Build history of the part. All positions in model axes, mm. A direction names the side the tool comes from. Coordinates: 2 decimals unless noted, no trailing zeros. Write each loop counter-clockwise with the first axis right and the second up, starting at its lowest first coordinate (ties: lowest second). Pieces come first, ordered by that corner, then holes.
```python
from build123d import *

# Parameters (mm, degrees)
EXTRUDE_1_DEPTH = 7.5


with BuildPart() as part:
    # 草图1 → 凸台-拉伸1 (new, symmetric)
    with BuildSketch(Plane.XY):
        with BuildLine():
            Line((0, 14.17), (937, 14.17))
            ThreePointArc((937, 14.17), (951.17, 0), (937, -14.17))
            Line((937, -14.17), (0, -14.17))
            ThreePointArc((0, -14.17), (-14.17, 0), (0, 14.17))
        make_face()
        with BuildLine():
            Line((0, 12.99), (937, 12.99))
            ThreePointArc((937, 12.99), (949.99, 0), (937, -12.99))
            Line((937, -12.99), (0, -12.99))
            ThreePointArc((0, -12.99), (-12.99, 0), (0, 12.99))
        make_face(mode=Mode.SUBTRACT)
    extrude(amount=EXTRUDE_1_DEPTH, both=True)


solid = part.part
```
1. Mould opens along Y. For faces 3 (the face through (462, 14.17, 0)), 4 (the face through (471, 14, 7.5)), 5 (the face through (475, -12.99, 0)) say: +Y half, -Y half, draft (parallel to the pull), parting line (faces both ways), or undercut.
Computed values:
face 3: +Y half
face 4: draft
face 5: undercut
2. Flat gauge pins, fed straight in: pin 1 (6 mm diameter, centred on y = -10, z = 4.5, fed in from +X); pin 2 (1.5 mm diameter, centred on y = 9, z = -3, fed in from +X); pin 3 (4 mm diameter, centred on y = -7.5, z = 2.5, fed in from +X). Where does each tip first touch, or does it go through?
Computed values:
pin 1: stops at x = 949.32
pin 2: stops at x = 948.52
pin 3: stops at x = 950.06
3. Saw through at C-C on z = 5. List the corners of the cut face in (x, y).
Computed values:
outline: (0, -14.17) - (937, -14.17) arc R14.17 ccw to (937, 14.17) - (0, 14.17) arc R14.17 ccw to start; hole (0, -12.99) - (937, -12.99) arc R12.99 ccw to (937, 12.99) - (0, 12.99) arc R12.99 ccw to start
4. Probe line 1 along Y through (x, z) = (281.5, 2); line 2 along X through (y, z) = (0.25, 6); line 3 along X through (y, z) = (11, -1.75). List the from-to ranges inside material, lowest first.
Computed values:
line 1: y = -14.17 to -12.99, 12.99 to 14.17
line 2: x = -14.17 to -12.99, 949.99 to 951.17
line 3: x = -8.93 to -6.91, 943.91 to 945.93
5. Saw through at A-A on y = 0. List the corners of the cut face in (x, z).
Computed values:
outline: (-14.17, -7.5) - (-12.99, -7.5) - (-12.99, 7.5) - (-14.17, 7.5) - close; (949.99, -7.5) - (951.17, -7.5) - (951.17, 7.5) - (949.99, 7.5) - close
6. 3-axis set-ups, long thin cutter, end or side, ignore diameter. For faces 1 (the face through (-12.987, -0.286, 0.105)), 2 (the face through (-14.167, -0.312, 0.105)): which of +Z, -Z, +X, -X, +Y, -Y reach the whole face in a straight line?
Computed values:
face 1: +Z, -Z
face 2: +Z, -Z, -X
7. Saw through at B-B on x = 245. List the corners of the cut face in (y, z).
Computed values:
outline: (-14.17, -7.5) - (-12.99, -7.5) - (-12.99, 7.5) - (-14.17, 7.5) - close; (12.99, -7.5) - (14.17, -7.5) - (14.17, 7.5) - (12.99, 7.5) - close
